The model under review builds one solid part; all positions refer to its coordinate system, in mm. A direction names the side the tool comes from. Round coordinates to 2 decimals unless told otherwise and drop trailing zeros. Loops run counter-clockwise (first coordinate to the right, second up) from the corner with the lowest first, then second, coordinate; pieces in that order, holes last. Notation, with made-up numbers: (29, 31) - (39, 31) arc R27 ccw to (39, 52) - close; hole circle Ø9 at (61.5, 5). An arc over 180 degrees is marked (long way). Answer as CSV lines item,"result".
from build123d import *

# Parameters (mm, degrees)
BOSS_EXTRUDE1_DEPTH = 45
SKETCH2_R           = 8
CUT_EXTRUDE1_DEPTH  = 134.914151605


with BuildPart() as part:
    # Sketch1 → Boss-Extrude1 (new body)
    with BuildSketch(Plane.XY):
        with BuildLine():
            Line((0, 0), (0, -117))
            ThreePointArc((0, -117), (1.464466094, -120.535533906), (5, -122))
            Line((5, -122), (27, -122))
            ThreePointArc((27, -122), (30.535533906, -120.535533906), (32, -117))
            Line((32, -117), (32, 0))
            Line((32, 0), (29, 0))
            Line((29, 0), (29, -117))
            ThreePointArc((29, -117), (28.414213562, -118.414213562), (27, -119))
            Line((27, -119), (5, -119))
            ThreePointArc((5, -119), (3.585786438, -118.414213562), (3, -117))
            Line((3, -117), (3, 0))
            Line((3, 0), (0, 0))
        make_face()
    extrude(amount=BOSS_EXTRUDE1_DEPTH)

    # Sketch2 → Cut-Extrude1 (cut, through all)
    with BuildSketch(Plane(origin=(32, 0, 0), x_dir=(0, 0, -1), z_dir=(1, 0, 0))):
        with Locations((-22.5, -12)):
            Circle(SKETCH2_R)
    extrude(amount=-CUT_EXTRUDE1_DEPTH, mode=Mode.SUBTRACT)


solid = part.part
1. Wall thickness on probe 1 along X at (y, z) = (-26, 4.5); probe 2 along Y at (x, z) = (6, 35); probe 3 along Y at (x, z) = (31.05, 22.5): over which ranges is each line inside the solid? List them lowest first.
Numbers:
probe 1,"x = 0 to 3, 29 to 32"
probe 2,"y = -122 to -119"
probe 3,"y = -119.93 to -20, -4 to 0"
2. Take a section at C-C (y = -12). State the section outline as (x, z) points, plus the area to 3 significant figures.
Numbers:
outline,"(0, 0) - (3, 0) - (3, 14.5) - (0, 14.5) - close; (0, 30.5) - (3, 30.5) - (3, 45) - (0, 45) - close; (29, 0) - (32, 0) - (32, 14.5) - (29, 14.5) - close; (29, 30.5) - (32, 30.5) - (32, 45) - (29, 45) - close"
area,"174 mm²"
3. Take a section at D-D (x = 23.5). State the section outline as (y, z) points.
Numbers:
outline,"(-122, 0) - (-119, 0) - (-119, 45) - (-122, 45) - close"
4. Take a section at A-A (z = 22.5). State the section outline as (x, y) points.
Numbers:
outline,"(0, -117) arc R5 ccw to (5, -122) - (27, -122) arc R5 ccw to (32, -117) - (32, -20) - (29, -20) - (29, -117) arc R2 cw to (27, -119) - (5, -119) arc R2 cw to (3, -117) - (3, -20) - (0, -20) - close; (0, -4) - (3, -4) - (3, 0) - (0, 0) - close; (29, -4) - (32, -4) - (32, 0) - (29, 0) - close"
5. Clearance check with flat-ended pins moving along their axes: pin 1 (9.5 mm diameter, centred on y = -12, z = 22.5, fed in from -X); pin 2 (6.5 mm diameter, centred on x = 12.5, z = 16, fed in from +Y). State where each tip first meets the part, or that it passes through.
Numbers:
pin 1,"passes through"
pin 2,"stops at y = -119"
6. Tool access review of faces 5 (the face through (3, -59, 22)), 6 (the face through (1.521, -16.868, 28.849)): name each direction out of +Z, -Z, +X, -X, +Y, -Y from which nothing blocks a thin tool from reaching the whole face with its end or side.
Numbers:
face 5,"+Z, -Z, +Y"
face 6,"+X, -X"
7. Draft analysis for pull direction Y (two halves, no side actions). For faces 1 (the face through (2, 0, 22)), 2 (the face through (1, -120, 22)), 3 (the face through (30.521, -16.868, 28.849)), 4 (the face through (2, -65, 0)), state which applies: +Y half, -Y half, draft (parallel to the pull), parting line (faces both ways), or undercut.
Numbers:
face 1,"+Y half"
face 2,"-Y half"
face 3,"undercut"
face 4,"draft"
8. Take a section at B-B (y = -36). State the section outline as (x, z) points, plus the area to 3 significant figures.
Numbers:
outline,"(0, 0) - (3, 0) - (3, 45) - (0, 45) - close; (29, 0) - (32, 0) - (32, 45) - (29, 45) - close"
area,"270 mm²"
